```python
from build123d import *

# Parameters (mm, degrees)
SWEEP_THIN1_PROFILE_R   = 15
SWEEP_THIN1_PROFILE_R_2 = 13


with BuildPart() as part:
    # Sweep-Thin1: sweep along a path in Sketch1
    with BuildLine(Plane.XY) as sweep_thin1_path:
        Line((500, 0), (40, 0))
        ThreePointArc((40, 0), (11.715728753, 11.715728753), (0, 40))
        Line((0, 40), (0, 600))
    # Sweep-Thin1 profile (on start of the path) → Sweep-Thin1 (sweep)
    with BuildSketch(Plane(origin=(500, 0, 0), x_dir=(0, 0, -1), z_dir=(-1, 0, 0))):
        Circle(SWEEP_THIN1_PROFILE_R)
        Circle(SWEEP_THIN1_PROFILE_R_2, mode=Mode.SUBTRACT)
    sweep(path=sweep_thin1_path.line)


solid = part.part
```
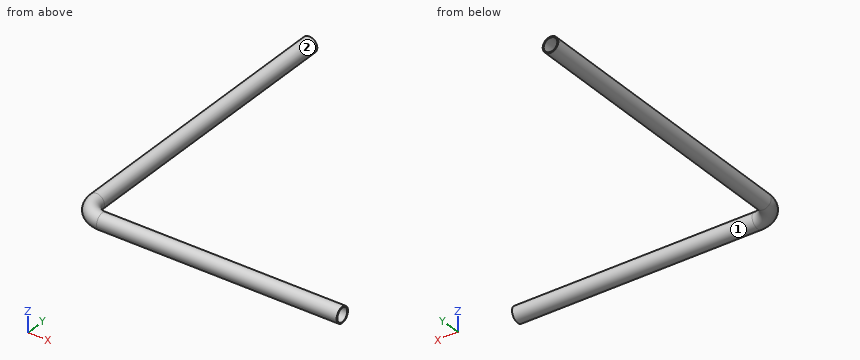
Part model, mm, in its own coordinate system. Face numbers are marked on the shaded views. A direction names the side the tool comes from. Round coordinates to 2 decimals unless told otherwise and drop trailing zeros. Loops run counter-clockwise (first coordinate to the right, second up) from the corner with the lowest first, then second, coordinate; pieces in that order, holes last. Notation, with made-up numbers: (13.5, 34) -> (22.5, 34) arc R23 cw to (22.5, 47) -> close; hole circle Ø5 at (72, -8). An arc over 180 degrees is marked (long way). Use CSV: the item, a comma, the result in double quotes. Start each with the question number.
1) Which spindle directions (+Z, -Z, +X, -X, +Y, -Y) get a long thin tool onto all of the face, cutting with end or side? Do the marked faces 1 and 2. Say none if no direction does.
2) Cut at A-A, the plane z = 0. Write the cut outline in (x, y), plus the area to 3 significant figures.
3) Wall check: L1, parallel to X at y = 268.5, z = -1; L2, parallel to Z at x = 182, y = 0; L3, parallel to Y at x = 268, z = 1.5. Give the ranges that are in metal, low to high. Write a range as [from, to].
4) Drop flat-ended pins along their axis: P1, Ø5, axis at y = 328, z = -8, coming from the -X side; P2, Ø4, axis at x = 42.5, z = 2, coming from the +Y side; P3, Ø15.5, axis at x = 0, z = 0, coming from the -Y side. Give the stop position or say it passes through.
5) Cut at B-B, the plane x = 246.5. Write the cut outline in (y, z).
Determined:
1,face 1,"+X"
1,face 2,"+Y"
2,outline,"(-15, 40) arc R55 ccw to (40, -15) -> (500, -15) -> (500, -13) -> (40, -13) arc R53 cw to (-13, 40) -> (-13, 600) -> (-15, 600) -> close; (13, 40) arc R27 ccw to (40, 13) -> (500, 13) -> (500, 15) -> (40, 15) arc R25 cw to (15, 40) -> (15, 600) -> (13, 600) -> close"
2,area,"4,330 mm2"
3,L1,"x = [-14.97, -12.96], [12.96, 14.97]"
3,L2,"z = [-15, -13], [13, 15]"
3,L3,"y = [-14.92, -12.91], [12.91, 14.92]"
4,P1,"stops at x = -13.96"
4,P2,"stops at y = 15"
4,P3,"stops at y = -4.55"
5,outline,"circle Ø30 at (0, 0); hole circle Ø26 at (0, 0)"
